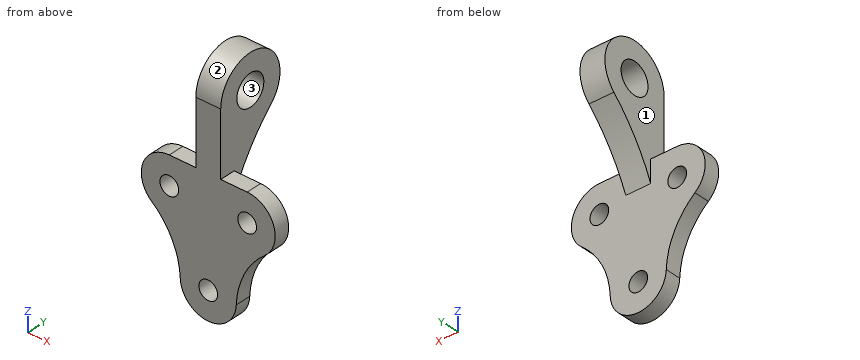
from build123d import *

# Parameters (mm, degrees)
BASE_PLATE_SKETCH_R = 6
BASE_PLATE_DEPTH    = 10
PIVOT_LUG_SKETCH_R  = 10
PIVOT_LUG_DEPTH     = 8


with BuildPart() as part:
    # Base Plate Sketch → Base Plate (new body)
    with BuildSketch(Plane(origin=(0, 0, 0), x_dir=(1, 0, 0), z_dir=(0, 1, 0))):
        with BuildLine():
            Line((25, -68), (8, -68))
            Line((8, -68), (8, -53.71))
            Line((8, -53.71), (-8, -53.71))
            Line((-8, -53.71), (-8, -68))
            Line((-8, -68), (-25, -68))
            ThreePointArc((-25, -68), (-41.958896227, -56.032896381), (-36.367918187, -36.043982083))
            ThreePointArc((-36.367918187, -36.043982083), (-23.224109156, -19.637945422), (-17.985565246, 0.720723799))
            ThreePointArc((-17.985565246, 0.720723799), (0, 18), (17.985565246, 0.720723799))
            ThreePointArc((17.985565246, 0.720723799), (23.224109156, -19.637945422), (36.367918187, -36.043982083))
            ThreePointArc((36.367918187, -36.043982083), (41.958896227, -56.032896381), (25, -68))
        make_face()
        with Locations(Location((0, 0, 0), (0, 0, 270))):
            Circle(BASE_PLATE_SKETCH_R, mode=Mode.SUBTRACT)
        with Locations(Location((-25, -50, 0), (0, 0, 270))):
            Circle(BASE_PLATE_SKETCH_R, mode=Mode.SUBTRACT)
        with Locations(Location((25, -50, 0), (0, 0, 270))):
            Circle(BASE_PLATE_SKETCH_R, mode=Mode.SUBTRACT)
    extrude(amount=BASE_PLATE_DEPTH)

    # Pivot Lug Sketch → Pivot Lug (add, symmetric)
    with BuildSketch(Plane(origin=(0, 0, 0), x_dir=(0, 0, -1), z_dir=(1, 0, 0))):
        with BuildLine():
            Line((-109, 0), (-53.71, 0))
            Line((-53.71, 0), (-53.71, 10))
            ThreePointArc((-53.71, 10), (-74.800840464, 21.756077977), (-93.237910195, 37.347850827))
            ThreePointArc((-93.237910195, 37.347850827), (-129.268851943, 30.554159275), (-109, 0))
        make_face()
        with Locations((-109, 22)):
            Circle(PIVOT_LUG_SKETCH_R, mode=Mode.SUBTRACT)
    extrude(amount=PIVOT_LUG_DEPTH, both=True)


solid = part.part
Work out the finished part from the listing and answer in its coordinate system (mm). Face numbers are marked on the shaded views. Coordinates: 2 decimals unless noted, no trailing zeros. Write each loop counter-clockwise with the first axis right and the second up, starting at its lowest first coordinate (ties: lowest second). Pieces come first, ordered by that corner, then holes.
1. For a pull along Y with two mould halves and no side action, classify the marked faces 1, 2 and 3 as +Y half, -Y half, draft (parallel to the pull), parting line (faces both ways), or undercut.
Results list:
face 1: draft
face 2: parting line
face 3: undercut
2. Flat-ended cylindrical pins translate along their axes: pin 1 (14 mm diameter, centred on x = 0, z = 0, fed in from +Y); pin 2 (8 mm diameter, centred on y = 38.5, z = 110, fed in from -X); pin 3 (8 mm diameter, centred on x = 18, y = 3, fed in from +Z). Find the tip coordinate at first contact, or state that the pin passes through.
Results list:
pin 1: stops at y = 10
pin 2: stops at x = -8
pin 3: stops at z = 68
3. The part is cut by section B-B, the plane z = 50. Write down the section's boundary in (x, y), and give its area (3 significant figures).
Results list:
outline: (-43, 0) - (-31, 0) - (-31, 10) - (-43, 10) - close; (-19, 0) - (19, 0) - (19, 10) - (-19, 10) - close; (31, 0) - (43, 0) - (43, 10) - (31, 10) - close
area: 620 mm2
4. Consider line 1 along X through (y, z) = (7, 50); line 2 along Y through (x, z) = (0.75, 109); line 3 along X through (y, z) = (23.5, 91.5). Determine where each line is inside the solid, lowest interval first.
Results list:
line 1: x = -43 to -31, -19 to 19, 31 to 43
line 2: y = 0 to 12, 32 to 44
line 3: x = -8 to 8
5. The part is cut by section A-A, the plane x = 0. Write down the section's boundary in (y, z), and give its area (3 significant figures).
Results list:
outline: (0, -18) - (10, -18) - (10, -6) - (0, -6) - close; (0, 6) - (10, 6) - (10, 53.71) arc R125 cw to (37.35, 93.24) arc R22 ccw (long way) to (0, 109) - close; hole circle Ø20 at (22, 109)
area: 2,570 mm2
6. The part is cut by section D-D, the plane x = 29.5. Write down the section's boundary in (y, z), and give its area (3 significant figures).
Results list:
outline: (0, 29.25) - (10, 29.25) - (10, 46.03) - (0, 46.03) - close; (0, 53.97) - (10, 53.97) - (10, 67.43) - (0, 67.43) - close
area: 302 mm2
7. The part is cut by section C-C, the plane y = 26. Write down the section's boundary in (x, z).
Results list:
outline: (-8, 80.57) - (8, 80.57) - (8, 99.83) - (-8, 99.83) - close; (-8, 118.17) - (8, 118.17) - (8, 130.63) - (-8, 130.63) - close
